Work out the finished part from the listing and answer in its coordinate system (mm). Face numbers are marked on the shaded views. Coordinates: 2 decimals unless noted, no trailing zeros. Order: outer loops, then holes, each group sorted by start corner. A loop starts at its lowest first (then second) coordinate and runs counter-clockwise, first axis right, second up.
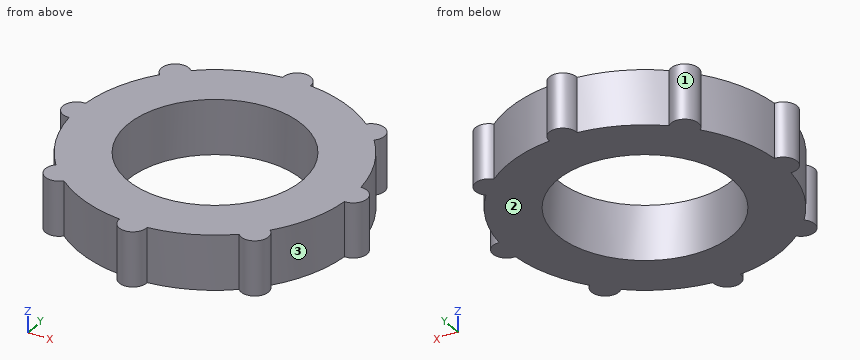
```python
from build123d import *

# Parameters (mm, degrees)
SKETCH_1_R      = 16
EXTRUDE_1_DEPTH = 10


with BuildPart() as part:
    # 草图1 → 凸台-拉伸1 (new body)
    with BuildSketch(Plane.XY):
        with BuildLine():
            ThreePointArc((-2.496873044, 24.875), (-9.567085809, 23.096988313), (-15.823725321, 19.354837043))
            ThreePointArc((-15.823725321, 19.354837043), (-19.445436483, 19.445436483), (-19.354837043, 15.823725321))
            ThreePointArc((-19.354837043, 15.823725321), (-23.096988313, 9.567085809), (-24.875, 2.496873044))
            ThreePointArc((-24.875, 2.496873044), (-27.5, 0), (-24.875, -2.496873044))
            ThreePointArc((-24.875, -2.496873044), (-23.096988313, -9.567085809), (-19.354837043, -15.823725321))
            ThreePointArc((-19.354837043, -15.823725321), (-19.445436483, -19.445436483), (-15.823725321, -19.354837043))
            ThreePointArc((-15.823725321, -19.354837043), (-9.567085809, -23.096988313), (-2.496873044, -24.875))
            ThreePointArc((-2.496873044, -24.875), (0, -27.5), (2.496873044, -24.875))
            ThreePointArc((2.496873044, -24.875), (9.567085809, -23.096988313), (15.823725321, -19.354837043))
            ThreePointArc((15.823725321, -19.354837043), (19.445436483, -19.445436483), (19.354837043, -15.823725321))
            ThreePointArc((19.354837043, -15.823725321), (23.096988313, -9.567085809), (24.875, -2.496873044))
            ThreePointArc((24.875, -2.496873044), (27.5, 0), (24.875, 2.496873044))
            ThreePointArc((24.875, 2.496873044), (23.096988313, 9.567085809), (19.354837043, 15.823725321))
            ThreePointArc((19.354837043, 15.823725321), (19.445436483, 19.445436483), (15.823725321, 19.354837043))
            ThreePointArc((15.823725321, 19.354837043), (9.567085809, 23.096988313), (2.496873044, 24.875))
            ThreePointArc((2.496873044, 24.875), (0, 27.5), (-2.496873044, 24.875))
        make_face()
        Circle(SKETCH_1_R, mode=Mode.SUBTRACT)
    extrude(amount=EXTRUDE_1_DEPTH)


solid = part.part
```
1. Flat-ended cylindrical pins translate along their axes: pin 1 (1.5 mm diameter, centred on x = -15.5, z = 3.5, fed in from +Y); pin 2 (12 mm diameter, centred on x = 12, y = 4.5, fed in from +Z); pin 3 (1.5 mm diameter, centred on x = 19, z = 4.5, fed in from -Y); pin 4 (6 mm diameter, centred on y = -7.5, z = 8.5, fed in from +X). Find the tip coordinate at first contact, or state that the pin passes through.
2. The part is cut by section A-A (z = 1.5). Determine the outline of the cut face in (x, y) (3 decimals).
3. The mould has two halves that part along X. Classify the marked faces 1, 2 and 3: released by +X, released by -X, zero draft, split by the parting line, or undercut.
4. Consider probe 1 along Y at (x, z) = (0, 7); probe 2 along Y at (x, z) = (-12.5, 2.25); probe 3 along X at (y, z) = (-6.5, 3.5). Determine where each line is inside the solid, lowest interval first.
5. The part is cut by section B-B (x = 0). Determine the outline of the cut face in (y, z), plus the area to 3 significant figures.
6. The part is cut by section C-C (y = 14.5). Determine the outline of the cut face in (x, z).
7. The part is cut by section D-D (y = -18). Determine the outline of the cut face in (x, z), plus the area to 3 significant figures.
Worked out:
1. pin 1: stops at y = 20.19
1. pin 2: stops at z = 10
1. pin 3: stops at y = -20.11
1. pin 4: stops at x = 24.59
2. outline: (-24.875, -2.497) arc R25 ccw to (-19.355, -15.824) arc R2.5 ccw (long way) to (-15.824, -19.355) arc R25 ccw to (-2.497, -24.875) arc R2.5 ccw (long way) to (2.497, -24.875) arc R25 ccw to (15.824, -19.355) arc R2.5 ccw (long way) to (19.355, -15.824) arc R25 ccw to (24.875, -2.497) arc R2.5 ccw (long way) to (24.875, 2.497) arc R25 ccw to (19.355, 15.824) arc R2.5 ccw (long way) to (15.824, 19.355) arc R25 ccw to (2.497, 24.875) arc R2.5 ccw (long way) to (-2.497, 24.875) arc R25 ccw to (-15.824, 19.355) arc R2.5 ccw (long way) to (-19.355, 15.824) arc R25 ccw to (-24.875, 2.497) arc R2.5 ccw (long way) to start; hole circle Ø32 at (0, 0)
3. face 1: undercut
3. face 2: zero draft
3. face 3: released by +X
4. probe 1: y = -27.5 to -16, 16 to 27.5
4. probe 2: y = -21.65 to -9.99, 9.99 to 21.65
4. probe 3: x = -24.14 to -14.62, 14.62 to 24.14
5. outline: (-27.5, 0) - (-16, 0) - (-16, 10) - (-27.5, 10) - close; (16, 0) - (27.5, 0) - (27.5, 10) - (16, 10) - close
5. area: 230 mm2
6. outline: (-20.37, 0) - (-6.76, 0) - (-6.76, 10) - (-20.37, 10) - close; (6.76, 0) - (20.37, 0) - (20.37, 10) - (6.76, 10) - close
7. outline: (-20.16, 0) - (20.16, 0) - (20.16, 10) - (-20.16, 10) - close
7. area: 403 mm2
